Design review of the part shown in the three views and the two pictorial views. Dimensions are in mm from the part's minimum x, y and z. A direction names the side the tool comes from. Give positions to 0.01 mm unless a question says otherwise; leave off trailing zeros. Loops run counter-clockwise (first coordinate to the right, second up) from the corner with the lowest first, then second, coordinate; pieces in that order, holes last.
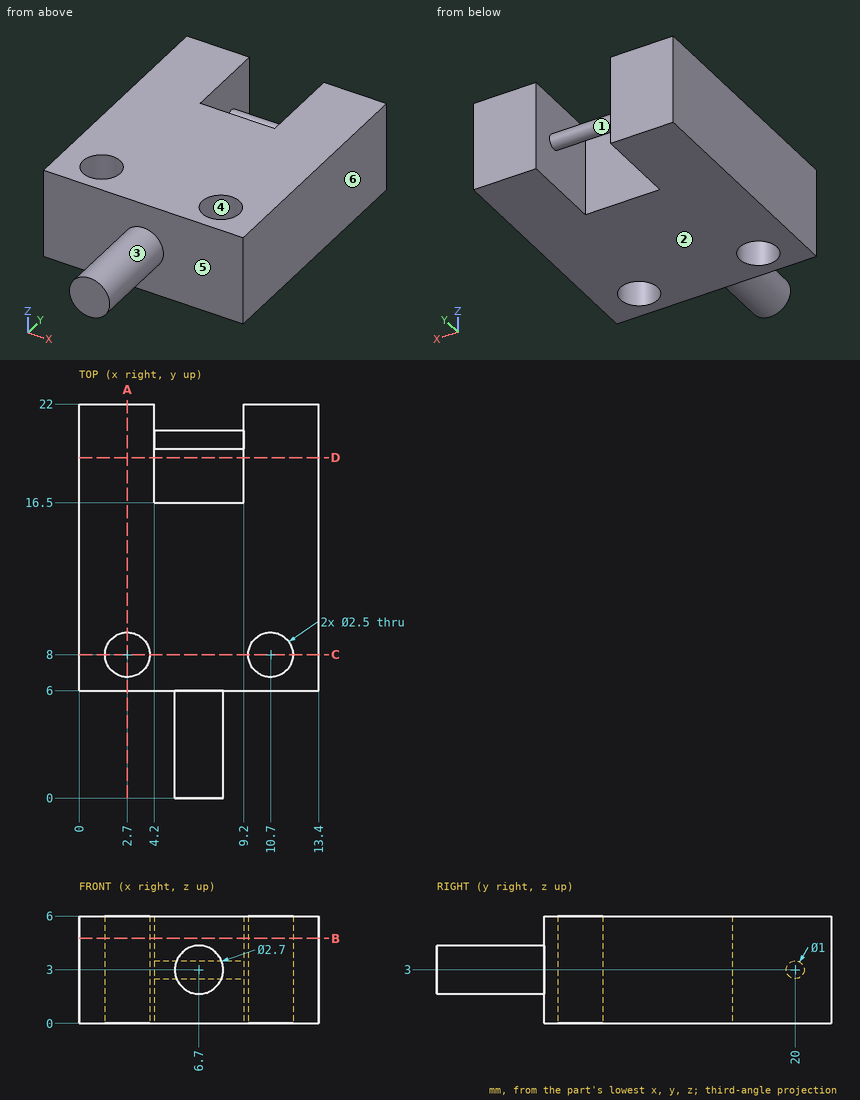
Q1. Mouldability with a two-part tool opening along Y and no side actions: class the marked faces 4, 5 and 6 as +Y half, -Y half, draft (parallel to the pull), parting line (faces both ways), or undercut.
Answers:
face 4: undercut
face 5: -Y half
face 6: draft
Q2. Consider section A-A on x = 2.7. Give the boundary of the cut face in (y, z).
Answers:
outline: (6, 0) - (6.75, 0) - (6.75, 6) - (6, 6) - close; (9.25, 0) - (22, 0) - (22, 6) - (9.25, 6) - close
Q3. Consider section D-D on y = 19. Give the boundary of the cut face in (x, z), plus the area to 3 significant figures.
Answers:
outline: (0, 0) - (4.2, 0) - (4.2, 6) - (0, 6) - close; (9.2, 0) - (13.4, 0) - (13.4, 6) - (9.2, 6) - close
area: 50.4 mm2
Q4. Consider section C-C on y = 8. Give the boundary of the cut face in (x, z), plus the area to 3 significant figures.
Answers:
outline: (0, 0) - (1.45, 0) - (1.45, 6) - (0, 6) - close; (3.95, 0) - (9.45, 0) - (9.45, 6) - (3.95, 6) - close; (11.95, 0) - (13.4, 0) - (13.4, 6) - (11.95, 6) - close
area: 50.4 mm2
Q5. Consider section B-B on z = 4.75. Give the boundary of the cut face in (x, y), plus the area to 3 significant figures.
Answers:
outline: (0, 6) - (13.4, 6) - (13.4, 22) - (9.2, 22) - (9.2, 16.5) - (4.2, 16.5) - (4.2, 22) - (0, 22) - close; hole circle Ø2.5 at (2.7, 8); hole circle Ø2.5 at (10.7, 8)
area: 177 mm2
Q6. For probe 1 along Y at (x, z) = (2.7, 4); probe 2 along X at (y, z) = (17, 5.75); probe 3 along Y at (x, z) = (13.25, 3.75), list the stretches that pass through material, from the lowest coordinate up.
Answers:
probe 1: y = 6 to 6.75, 9.25 to 22
probe 2: x = 0 to 4.2, 9.2 to 13.4
probe 3: y = 6 to 22
Q7. For pin 1 Ø1.5 at (x, z) = (6.5, 3.5) entering from +Y, flat-tipped, find the tip position at first contact; note if it passes through.
Answers:
pin 1: stops at y = 20.5
Q8. Machinability: for the marked faces 1, 2 and 3, which of the approach directions +Z, -Z, +X, -X, +Y, -Y give a long, thin tool a straight path to every point of the face, cutting with its end or side? Answer none if there is none.
Answers:
face 1: none
face 2: -Z, +X, -X, +Y, -Y
face 3: -Y
